Build history of the part. All positions in model axes, mm. Face numbers are marked on the shaded views. A direction names the side the tool comes from. Round coordinates to 2 decimals unless told otherwise and drop trailing zeros. Write each loop counter-clockwise with the first axis right and the second up, starting at its lowest first coordinate (ties: lowest second). Pieces come first, ordered by that corner, then holes. Notation, with made-up numbers: (62, 86) -> (104, 86) arc R7 ccw to (104, 96) -> close; hole circle Ø5 at (-5.5, 87). An arc over 180 degrees is marked (long way). Answer in a Markdown table with one row per item.
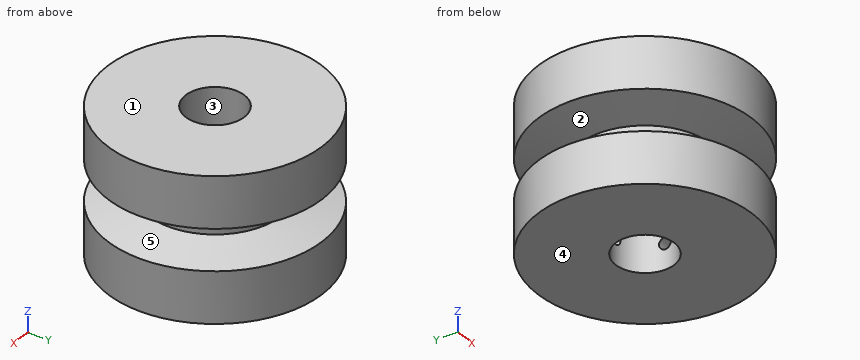
```python
from build123d import *

# Parameters (mm, degrees)
SKETCH_1_R      = 37.5
SKETCH_1_R_2    = 10.25
EXTRUDE_1_DEPTH = 50


with BuildPart() as part:
    # 草图1 → 凸台-拉伸1 (new body)
    with BuildSketch(Plane.XY):
        Circle(SKETCH_1_R)
        Circle(SKETCH_1_R_2, mode=Mode.SUBTRACT)
    extrude(amount=EXTRUDE_1_DEPTH)

    # 草图2 → 切除-旋转1 (revolve, cut)
    with BuildSketch(Plane(origin=(0, 0, 0), x_dir=(1, 0, 0), z_dir=(0, 1, 0))):
        Polygon((-38.25, -17.648818614), (-23.25, -21.25), (-23.25, -28.75), (-38.25, -32.351181386), align=None)
    revolve(axis=Axis((0, 0, 0), (0, 0, 1)), mode=Mode.SUBTRACT)

    # 草图3 → M5 螺纹孔2 (revolve, cut)
    with BuildSketch(Plane(origin=(0, 32.5, 9), x_dir=(0, 0, 1), z_dir=(1, 0, 0))):
        Polygon((0, 0), (0, 31.2618073), (2.1, 30), (2.1, 0), align=None)
    revolve(axis=Axis((0, 38.85, 9), (0, -1, 0)), mode=Mode.SUBTRACT)

    # 草图5 → M5 螺纹孔1 (revolve, cut)
    with BuildSketch(Plane(origin=(32.5, 0, 9), x_dir=(0, 0, -1), z_dir=(0, 1, 0))):
        Polygon((0, 0), (0, 31.2618073), (2.1, 30), (2.1, 0), align=None)
    revolve(axis=Axis((38.85, 0, 9), (-1, 0, 0)), mode=Mode.SUBTRACT)


solid = part.part
```
Q1. Drop flat-ended pins along their axis: P1, Ø4, axis at y = 22.5, z = 9, coming from the -X side; P2, Ø6.5, axis at x = 0, z = 9, coming from the +Y side; P3, Ø1.3, axis at x = 1, z = 9.5, coming from the -Y side. Give the stop position or say it passes through.
A:
| item | result |
|---|---|
| P1 | x = -31.4 |
| P2 | y = 37.5 |
| P3 | y = -37.5 |
Q2. Which spindle directions (+Z, -Z, +X, -X, +Y, -Y) get a long thin tool onto all of the face, cutting with end or side? Do the marked faces 1 and 2. Say none if no direction does.
A:
| item | result |
|---|---|
| face 1 | +Z, +X, -X, +Y, -Y |
| face 2 | none |
Q3. Saw through at A-A on x = 0. Write the cut outline in (y, z).
A:
| item | result |
|---|---|
| outline | (-37.5, 0) -> (-10.25, 0) -> (-10.25, 50) -> (-37.5, 50) -> (-37.5, 32.17) -> (-23.25, 28.75) -> (-23.25, 21.25) -> (-37.5, 17.83) -> close; (10.25, 0) -> (37.5, 0) -> (37.5, 17.83) -> (23.25, 21.25) -> (23.25, 28.75) -> (37.5, 32.17) -> (37.5, 50) -> (10.25, 50) -> (10.25, 11.1) -> (32.5, 11.1) -> (32.5, 6.9) -> (10.25, 6.9) -> close |
Q4. Two-plate mould, pull along Y, no slides. Class the marked faces 3, 4 and 5: released by +Y, released by -Y, zero draft, split by the parting line, or undercut.
A:
| item | result |
|---|---|
| face 3 | undercut |
| face 4 | zero draft |
| face 5 | split by the parting line |
Q5. Wall check: line 1 (Y direction, x = 0, z = 36); line 2 (Z direction, x = 17, y = 0); line 3 (X direction, y = 7, z = 28). Give the ranges that are in metal, low to high. Write a range as [from, to].
A:
| item | result |
|---|---|
| line 1 | [-37.5, -10.25], [10.25, 37.5] |
| line 2 | [0, 6.9], [11.1, 50] |
| line 3 | [-22.17, -7.49], [7.49, 22.17] |
Q6. Saw through at D-D on y = 26. State how many separate pieces and enclosed holes the cut face has, plus the area to 3 significant figures.
A:
| item | result |
|---|---|
| separate pieces | 2 |
| enclosed holes | 1 |
| area | 2,100 mm² |
Q7. Saw through at C-C on z = 9. Write the cut outline in (x, y), plus the area to 3 significant figures.
A:
| item | result |
|---|---|
| outline | circle Ø75 at (0, 0); hole (-2.1, 10.03) arc R10.25 ccw (long way) to (10.03, -2.1) -> (32.5, -2.1) -> (32.5, 2.1) -> (10.03, 2.1) arc R10.25 ccw to (2.1, 10.03) -> (2.1, 32.5) -> (-2.1, 32.5) -> close |
| area | 3,900 mm² |
